CAD build for the part. Positions are in the model's coordinates, mm. A direction names the side the tool comes from. Round coordinates to 2 decimals unless told otherwise and drop trailing zeros. Loops run counter-clockwise (first coordinate to the right, second up) from the corner with the lowest first, then second, coordinate; pieces in that order, holes last.
```python
from build123d import *

# Parameters (mm, degrees)
BOSS_EXTRUDE1_DEPTH                          = 10
SKETCH2_R                                    = 40
BOSS_EXTRUDE2_DEPTH                          = 20
SKETCH3_R                                    = 3
CBORE_FOR_M6_HEXAGON_SOCKET_HEAD_CAP_2_COUNT = 2
CBORE_FOR_M6_HEXAGON_SOCKET_HEAD_CAP_2_PITCH = 80
CBORE_FOR_M6_HEXAGON_SOCKET_HEAD_CAP_3_COUNT = 2
CBORE_FOR_M6_HEXAGON_SOCKET_HEAD_CAP_3_PITCH = 100
CBORE_FOR_M6_HEXAGON_SOCKET_HEAD_CAP_4_COUNT = 2
CBORE_FOR_M6_HEXAGON_SOCKET_HEAD_CAP_4_PITCH = 60
SKETCH4_R                                    = 7.5
BOSS_EXTRUDE3_DEPTH                          = 25
CHAMFER1_SIZE                                = 1
SKETCH5_R                                    = 45
CUT_EXTRUDE1_DEPTH                           = 2


with BuildPart() as part:
    # Sketch1 → Boss-Extrude1 (new body)
    with BuildSketch(Plane(origin=(0, 0, 0), x_dir=(1, 0, 0), z_dir=(0, 1, 0))):
        with BuildLine():
            Line((-43, 50), (43, 50))
            ThreePointArc((43, 50), (55.02081528, 45.02081528), (60, 33))
            Line((60, 33), (60, -33))
            ThreePointArc((60, -33), (55.02081528, -45.02081528), (43, -50))
            Line((43, -50), (-43, -50))
            ThreePointArc((-43, -50), (-55.02081528, -45.02081528), (-60, -33))
            Line((-60, -33), (-60, 33))
            ThreePointArc((-60, 33), (-55.02081528, 45.02081528), (-43, 50))
        make_face()
    extrude(amount=BOSS_EXTRUDE1_DEPTH)

    # Sketch2 → Boss-Extrude2 (add)
    with BuildSketch(Plane.XZ):
        with Locations(Location((0, 0, 0), (0, 0, 270))):
            Circle(SKETCH2_R)
    extrude(amount=BOSS_EXTRUDE2_DEPTH)

    # Sketch3 → Revolve1 (revolve)
    with BuildSketch(Plane(origin=(0, 0, 0), x_dir=(0, 0, -1), z_dir=(1, 0, 0)), mode=Mode.PRIVATE) as revolve1_sk:
        with Locations((-40, -17)):
            Circle(SKETCH3_R)
    revolve(revolve1_sk.sketch.rotate(Axis((0, 22.515244343, 0), (0, -1, 0)), 180), axis=Axis((0, 22.515244343, 0), (0, -1, 0)))

    # Sketch9 → CBORE for M6 Hexagon socket head cap screws1 (revolve, cut)
    with BuildSketch(Plane(origin=(-40, 10, -30), x_dir=(0, 0, 1), z_dir=(1, 0, 0))):
        Polygon((0, 0), (0, 30), (3.3, 30), (3.3, 6.8), (5.5, 6.8), (5.5, 0.025), (5.525, 0), align=None)
    cbore_for_m6_hexagon_socket_head_cap_scr = revolve(axis=Axis((-40, 16.35, -30), (0, -1, 0)), mode=Mode.SUBTRACT)

    # CBORE for M6 Hexagon socket head cap 2: CBORE for M6 Hexagon socket head cap screws1 ×2
    with Locations(*[(i * CBORE_FOR_M6_HEXAGON_SOCKET_HEAD_CAP_2_PITCH, 0, 0) for i in range(1, CBORE_FOR_M6_HEXAGON_SOCKET_HEAD_CAP_2_COUNT)]):
        add(cbore_for_m6_hexagon_socket_head_cap_scr, mode=Mode.SUBTRACT)

    # CBORE for M6 Hexagon socket head cap 3: CBORE for M6 Hexagon socket head cap screws1 ×2
    with Locations(*[Vector(0.7999999999999999, 0, 0.6000000000000001) * (i * CBORE_FOR_M6_HEXAGON_SOCKET_HEAD_CAP_3_PITCH) for i in range(1, CBORE_FOR_M6_HEXAGON_SOCKET_HEAD_CAP_3_COUNT)]):
        add(cbore_for_m6_hexagon_socket_head_cap_scr, mode=Mode.SUBTRACT)

    # CBORE for M6 Hexagon socket head cap 4: CBORE for M6 Hexagon socket head cap screws1 ×2
    with Locations(*[(0, 0, i * CBORE_FOR_M6_HEXAGON_SOCKET_HEAD_CAP_4_PITCH) for i in range(1, CBORE_FOR_M6_HEXAGON_SOCKET_HEAD_CAP_4_COUNT)]):
        add(cbore_for_m6_hexagon_socket_head_cap_scr, mode=Mode.SUBTRACT)

    # Sketch4 → Boss-Extrude3 (add)
    with BuildSketch(Plane.XZ.offset(20)):
        with Locations(Location((0, 0, 0), (0, 0, 270))):
            Circle(SKETCH4_R)
    extrude(amount=BOSS_EXTRUDE3_DEPTH)

    # Chamfer1
    chamfer1_edges = [part.edges().sort_by_distance(p)[0] for p in [
        (0, -45, 7.5),
    ]]
    chamfer(chamfer1_edges, length=CHAMFER1_SIZE)

    # Sketch5 → Cut-Extrude1 (cut)
    with BuildSketch(Plane(origin=(0, 10, 0), x_dir=(1, 0, 0), z_dir=(0, 1, 0))):
        Circle(SKETCH5_R)
    extrude(amount=-CUT_EXTRUDE1_DEPTH, mode=Mode.SUBTRACT)


solid = part.part
```
Item 1: Cut at C-C, the plane x = 0. Give the cut face in (y, z).
Answers follow:
outline: (-45, -6.5) - (-44, -7.5) - (-20, -7.5) - (-20, -40) arc R3 ccw to (-14, -40) - (0, -40) - (0, -50) - (10, -50) - (10, -45) - (8, -45) - (8, 45) - (10, 45) - (10, 50) - (0, 50) - (0, 40) - (-14, 40) arc R3 ccw to (-20, 40) - (-20, 7.5) - (-44, 7.5) - (-45, 6.5) - close
Item 2: Cut at B-B, the plane z = 0. Give the cut face in (x, y).
Answers follow:
outline: (-60, 0) - (-40, 0) - (-40, -14) arc R3 ccw to (-40, -20) - (-7.5, -20) - (-7.5, -44) - (-6.5, -45) - (6.5, -45) - (7.5, -44) - (7.5, -20) - (40, -20) arc R3 ccw to (40, -14) - (40, 0) - (60, 0) - (60, 10) - (45, 10) - (45, 8) - (-45, 8) - (-45, 10) - (-60, 10) - close
Item 3: 3-axis set-ups, long thin cutter, end or side, ignore diameter. For faces 4 (the flat face through (41, 0, -1)), 5 (the flat face through (-60, 5, 0)), 6 (the cylindrical face through (-0.554, 9.014, 44.997)): which of +Z, -Z, +X, -X, +Y, -Y reach the whole face in a straight line?
Answers follow:
face 4: none
face 5: +Z, -Z, -X, +Y, -Y
face 6: +Y
Item 4: Probe line 1 (Z direction, x = 40, y = 4.5); line 2 (X direction, y = 4.5, z = 30); line 3 (X direction, y = 2.4, z = 30). List the from-to ranges inside material, lowest first.
Answers follow:
line 1: z = -50 to -35.5, -24.5 to 24.5, 35.5 to 50
line 2: x = -60 to -45.5, -34.5 to 34.5, 45.5 to 60
line 3: x = -60 to -43.3, -36.7 to 36.7, 43.3 to 60
Item 5: Cut at A-A, the plane y = 5.5. Give the cut face in (x, z), plus the area to 3 significant figures.
Answers follow:
outline: (-60, -33) arc R17 ccw to (-43, -50) - (43, -50) arc R17 ccw to (60, -33) - (60, 33) arc R17 ccw to (43, 50) - (-43, 50) arc R17 ccw to (-60, 33) - close; hole circle Ø11 at (-40, -30); hole circle Ø11 at (-40, 30); hole circle Ø11 at (40, -30); hole circle Ø11 at (40, 30)
area: 11,400 mm2
Item 6: Flat gauge pins, fed straight in: P1, Ø1, axis at x = -39, z = -16, coming from the +Y side; P2, Ø4, axis at y = -7.5, z = 33.5, coming from the -X side; P3, Ø4, axis at x = -40, z = 30, coming from the +Y side; P4, Ø17.5, axis at x = 40, z = 30, coming from the -Y side. Where does each tip first touch, or does it go through?
Answers follow:
P1: stops at y = 8
P2: stops at x = -24.65
P3: passes through
P4: stops at y = -19.73
Item 7: Cut at D-D, the plane y = -5. Give the cut face in (x, z).
Answers follow:
outline: circle Ø80 at (0, 0)
Item 8: Two-plate mould, pull along Z, no slides. Class faces 1 (the flat face through (40, 3.2, -34)), 2 (the flat face through (1, -20, -8)), 3 (the cylindrical face through (55.15, 4.93, 44.89)): released by +Z, released by -Z, zero draft, split by the parting line, or undercut.
Answers follow:
face 1: undercut
face 2: zero draft
face 3: released by +Z
